Read the model definition and answer for the solid it produces. Units are mm, in the model's axes. A direction names the side the tool comes from. Give positions to 0.01 mm unless a question says otherwise; leave off trailing zeros. Order: outer loops, then holes, each group sorted by start corner. A loop starts at its lowest first (then second) coordinate and runs counter-clockwise, first axis right, second up.
```python
from build123d import *

# Parameters (mm, degrees)
BOSS_EXTRUDE1_DEPTH = 340
CUT_EXTRUDE1_DEPTH  = 409.809246471


with BuildPart() as part:
    # Sketch1 → Boss-Extrude1 (new, symmetric)
    with BuildSketch(Plane(origin=(0, 0, 0), x_dir=(0, 0, -1), z_dir=(1, 0, 0))):
        with BuildLine():
            Line((25, -50), (25, 50))
            Line((25, 50), (30, 222.99103121))
            ThreePointArc((30, 222.99103121), (0, 225), (-30, 222.99103121))
            Line((-30, 222.99103121), (-25, 50))
            Line((-25, 50), (-25, -50))
            Line((-25, -50), (-30, -222.99103121))
            ThreePointArc((-30, -222.99103121), (0, -225), (30, -222.99103121))
            Line((30, -222.99103121), (25, -50))
        make_face()
    extrude(amount=BOSS_EXTRUDE1_DEPTH, both=True)

    # Sketch2 → Cut-Extrude1 (cut, symmetric)
    with BuildSketch(Plane.XY):
        with BuildLine():
            Line((-145, -70), (-195, -70))
            ThreePointArc((-195, -70), (-219.748737342, -59.748737342), (-230, -35))
            Line((-230, -35), (-230, 35))
            ThreePointArc((-230, 35), (-219.748737342, 59.748737342), (-195, 70))
            Line((-195, 70), (-145, 70))
            ThreePointArc((-145, 70), (-120.251262658, 59.748737342), (-110, 35))
            Line((-110, 35), (-110, -35))
            ThreePointArc((-110, -35), (-120.251262658, -59.748737342), (-145, -70))
        make_face()
    cut_extrude1 = extrude(amount=CUT_EXTRUDE1_DEPTH, both=True, mode=Mode.SUBTRACT)

    # Mirror1: Cut-Extrude1 across plane
    add(cut_extrude1.mirror(Plane(origin=(0, 0, 0), x_dir=(0, 0, 1), z_dir=(1, 0, 0))), mode=Mode.SUBTRACT)


solid = part.part
```
1) The part is cut by section A-A on x = -178.5. Determine the outline of the cut face in (y, z), and give its area (3 significant figures).
Final values:
outline: (-222.99, -30) - (-70, -25.58) - (-70, 25.58) - (-222.99, 30) arc R225 ccw to start; (70, -25.58) - (222.99, -30) arc R225 ccw to (222.99, 30) - (70, 25.58) - close
area: 17,200 mm2
2) The part is cut by section D-D on x = 53.5. Determine the outline of the cut face in (y, z).
Final values:
outline: (-222.99, -30) - (-50, -25) - (50, -25) - (222.99, -30) arc R225 ccw to (222.99, 30) - (50, 25) - (-50, 25) - (-222.99, 30) arc R225 ccw to start
3) Given pin 1 (1 mm diameter, centred on x = -201, y = -98.5, fed in from +Z); pin 2 (15 mm diameter, centred on x = 175, z = -12.5, fed in from +Y); pin 3 (6 mm diameter, centred on x = -131.5, y = -103.5, fed in from -Z), each flat-ended and moving along its own axis, determine where each tip first touches the part or whether it passes through.
Final values:
pin 1: stops at z = 26.42
pin 2: stops at y = 224.94
pin 3: stops at z = -26.63
4) Consider L1, parallel to Y at x = 151, z = 8; L2, parallel to Y at x = 16.5, z = 5; L3, parallel to Y at x = 238, z = -2. Determine where each line is inside the solid, lowest interval first.
Final values:
L1: y = -224.86 to -70, 70 to 224.86
L2: y = -224.94 to 224.94
L3: y = -224.99 to 224.99
5) A tool of negligible diameter and unlimited length cuts with its end or side. For faces 3 (the face through (-283, -1, -25)), 4 (the face through (2, 1, 25)), 5 (the face through (119.981, -59.475, 0.358)), from which of +Z, -Z, +X, -X, +Y, -Y can it reach the whole face along a straight path? Write none if from no direction.
Final values:
face 3: -Z, +X, -X
face 4: +Z, +X, -X
face 5: +Z, -Z
6) The part is cut by section B-B on y = 25.5. Determine the outline of the cut face in (x, z).
Final values:
outline: (-340, -25) - (-230, -25) - (-230, 25) - (-340, 25) - close; (-110, -25) - (110, -25) - (110, 25) - (-110, 25) - close; (230, -25) - (340, -25) - (340, 25) - (230, 25) - close
7) The part is cut by section C-C on z = 15.5. Determine the outline of the cut face in (x, y), and give its area (3 significant figures).
Final values:
outline: (-340, -224.47) - (340, -224.47) - (340, 224.47) - (-340, 224.47) - close; hole (-230, -35) arc R35 ccw to (-195, -70) - (-145, -70) arc R35 ccw to (-110, -35) - (-110, 35) arc R35 ccw to (-145, 70) - (-195, 70) arc R35 ccw to (-230, 35) - close; hole (110, -35) arc R35 ccw to (145, -70) - (195, -70) arc R35 ccw to (230, -35) - (230, 35) arc R35 ccw to (195, 70) - (145, 70) arc R35 ccw to (110, 35) - close
area: 274,000 mm2
8) For a pull along Y with two mould halves and no side action, classify faces 1 (the face through (-230, 0, 0)), 2 (the face through (-340, 3, 0)) as released by +Y, released by -Y, zero draft, split by the parting line, or undercut.
Final values:
face 1: undercut
face 2: zero draft
